Could you check a few things on this model? Use its own coordinates, in mm. A direction names the side the tool comes from. Give positions to 0.01 mm unless a question says otherwise; leave off trailing zeros. Order: outer loops, then holes, each group sorted by start corner. A loop starts at its lowest first (then second) coordinate and runs counter-clockwise, first axis right, second up. Notation, with made-up numbers: (63, 12) -> (83, 12) arc R18 cw to (83, 26) -> close; hole circle Ø5 at (19, -16). An arc over 180 degrees is marked (long way). One line per item, written item: value.
```python
from build123d import *

# Parameters (mm, degrees)
SKETCH2_R          = 1.5
CUT_EXTRUDE1_DEPTH = 67.520673478


with BuildPart() as part:
    # Sketch1 → Revolve1 (revolve)
    with BuildSketch(Plane.XY, mode=Mode.PRIVATE) as revolve1_sk:
        with BuildLine():
            Line((-40, 0), (-30, 0))
            Line((-30, 0), (-30, 5))
            ThreePointArc((-30, 5), (-21.213203436, 26.213203436), (0, 35))
            Line((0, 35), (0, 36.5))
            ThreePointArc((0, 36.5), (-22.273863607, 27.273863607), (-31.5, 5))
            Line((-31.5, 5), (-31.5, 1.5))
            Line((-31.5, 1.5), (-40, 1.5))
            Line((-40, 1.5), (-40, 0))
        make_face()
    revolve(revolve1_sk.sketch.rotate(Axis((0, 35, 0), (0, 1, 0)), 180), axis=Axis((0, 35, 0), (0, 1, 0)))

    # Sketch2 → Cut-Extrude1 (cut, through all)
    with BuildSketch(Plane(origin=(0, 1.5, 0), x_dir=(1, 0, 0), z_dir=(0, 1, 0))):
        with Locations(Location((-35, 0, 0), (0, 0, 180))):
            Circle(SKETCH2_R)
        with Locations(Location((-17.5, 30.310889132, 0), (0, 0, 180))):
            Circle(SKETCH2_R)
        with Locations(Location((17.5, 30.310889132, 0), (0, 0, 180))):
            Circle(SKETCH2_R)
        with Locations(Location((35, 0, 0), (0, 0, 180))):
            Circle(SKETCH2_R)
        with Locations(Location((17.5, -30.310889132, 0), (0, 0, 180))):
            Circle(SKETCH2_R)
        with Locations(Location((-17.5, -30.310889132, 0), (0, 0, 180))):
            Circle(SKETCH2_R)
    extrude(amount=-CUT_EXTRUDE1_DEPTH, mode=Mode.SUBTRACT)


solid = part.part
```
1) Suppose I cut it at A-A, the plane z = 0. Write out the boundary of the cut face in (x, y), then the cut area to 3 significant figures.
Answer below:
outline: (-40, 0) -> (-36.5, 0) -> (-36.5, 1.5) -> (-40, 1.5) -> close; (-33.5, 0) -> (-30, 0) -> (-30, 5) arc R30 cw to (30, 5) -> (30, 0) -> (33.5, 0) -> (33.5, 1.5) -> (31.5, 1.5) -> (31.5, 5) arc R31.5 ccw to (-31.5, 5) -> (-31.5, 1.5) -> (-33.5, 1.5) -> close; (36.5, 0) -> (40, 0) -> (40, 1.5) -> (36.5, 1.5) -> close
area: 176 mm2
2) For faces 4 (the flat face through (21, 1.5, -24)), 5 (the cylindrical face through (16.128, 2.535, -25.296)), 6 (the cylindrical face through (36.2, 0.8, -0.9)), which set-ups out of +Z, -Z, +X, -X, +Y, -Y let a thin tool reach every point of the face, with its end or its side?
Answer below:
face 4: +Y
face 5: -Y
face 6: +Y, -Y
3) For P1, Ø8, axis at x = 4.5, y = 9, coming from the +Z side; P2, Ø2.5, axis at x = 35, z = 0, coming from the +Y side; P3, Ø3.5, axis at x = -35, z = 0, coming from the +Y side; P4, Ø5, axis at x = 11, y = 25, coming from the -Z side, each with a flat end and sliding along its axis, tell me the tip position at first contact or that it passes through.
Answer below:
P1: stops at z = 31.44
P2: passes through
P3: stops at y = 1.5
P4: stops at z = -24.07
4) If I drill on line 1 along Z through (x, y) = (0, 1.1); line 2 along Z through (x, y) = (17.5, 0.95); line 3 along Z through (x, y) = (35, 0.6), over which ranges is the centre line in solid material (lowest first)?
Answer below:
line 1: z = -40 to -30, 30 to 40
line 2: z = -35.97 to -31.81, -28.81 to -24.37, 24.37 to 28.81, 31.81 to 35.97
line 3: z = -19.36 to -1.5, 1.5 to 19.36
5) Suppose I cut it at C-C, the plane x = 0. Write out the boundary of the cut face in (y, z), then the cut area to 3 significant figures.
Answer below:
outline: (0, -40) -> (1.5, -40) -> (1.5, -31.5) -> (5, -31.5) arc R31.5 ccw to (5, 31.5) -> (1.5, 31.5) -> (1.5, 40) -> (0, 40) -> (0, 30) -> (5, 30) arc R30 cw to (5, -30) -> (0, -30) -> close
area: 185 mm2
6) We'd pull the mould along Z, two halves only. Please class faces 1 (the cylindrical face through (18.61, 0.76, -29.3)), 2 (the cylindrical face through (-4.101, 3.226, -31.232)), 3 (the flat face through (-15, 0, 26.5)): +Z half, -Z half, draft (parallel to the pull), parting line (faces both ways), or undercut.
Answer below:
face 1: undercut
face 2: parting line
face 3: draft
7) Suppose I cut it at B-B, the plane x = 35. Write out the boundary of the cut face in (y, z), then the cut area to 3 significant figures.
Answer below:
outline: (0, -19.36) -> (1.5, -19.36) -> (1.5, -1.5) -> (0, -1.5) -> close; (0, 1.5) -> (1.5, 1.5) -> (1.5, 19.36) -> (0, 19.36) -> close
area: 53.6 mm2
8) Suppose I cut it at D-D, the plane x = -17.5. Write out the boundary of the cut face in (y, z).
Answer below:
outline: (0, -35.97) -> (1.5, -35.97) -> (1.5, -31.81) -> (0, -31.81) -> close; (0, -28.81) -> (1.5, -28.81) -> (1.5, -26.19) -> (5, -26.19) arc R26.19 ccw to (5, 26.19) -> (1.5, 26.19) -> (1.5, 28.81) -> (0, 28.81) -> (0, 24.37) -> (5, 24.37) arc R24.37 cw to (5, -24.37) -> (0, -24.37) -> close; (0, 31.81) -> (1.5, 31.81) -> (1.5, 35.97) -> (0, 35.97) -> close
